The figure shows three views and two pictorial views of one solid part (mm, origin at its lowest corner). Answer the questions. Coordinates: 2 decimals unless noted, no trailing zeros. Loops run counter-clockwise (first coordinate to the right, second up) from the corner with the lowest first, then second, coordinate; pieces in that order, holes last. Notation, with made-up numbers: (46, 76) - (56, 76) arc R16 cw to (56, 81) - close; hole circle Ø8 at (0, 71.25). An arc over 180 degrees is marked (long way). Return JSON: item names as keys, results as strings. Group by question number.
1. This flat-tipped pin is pushed along its axis until it touches: P1, Ø4, axis at x = 40, y = 50, coming from the -Z side. Where does it stop, or does it pass through?
2. Section A-A (y = 5.3) is taken. Write down the section's boundary in (x, z), and give its area (3 significant figures).
3. Section B-B (x = 22.25) is taken. Write down the section's boundary in (y, z).
4. Find the intervals of material crossed by line 1 along Y through (x, z) = (22.25, 19.5); line 2 along X through (y, z) = (52.7, 18.75); line 3 along Y through (x, z) = (23, 15.5), in increasing order.
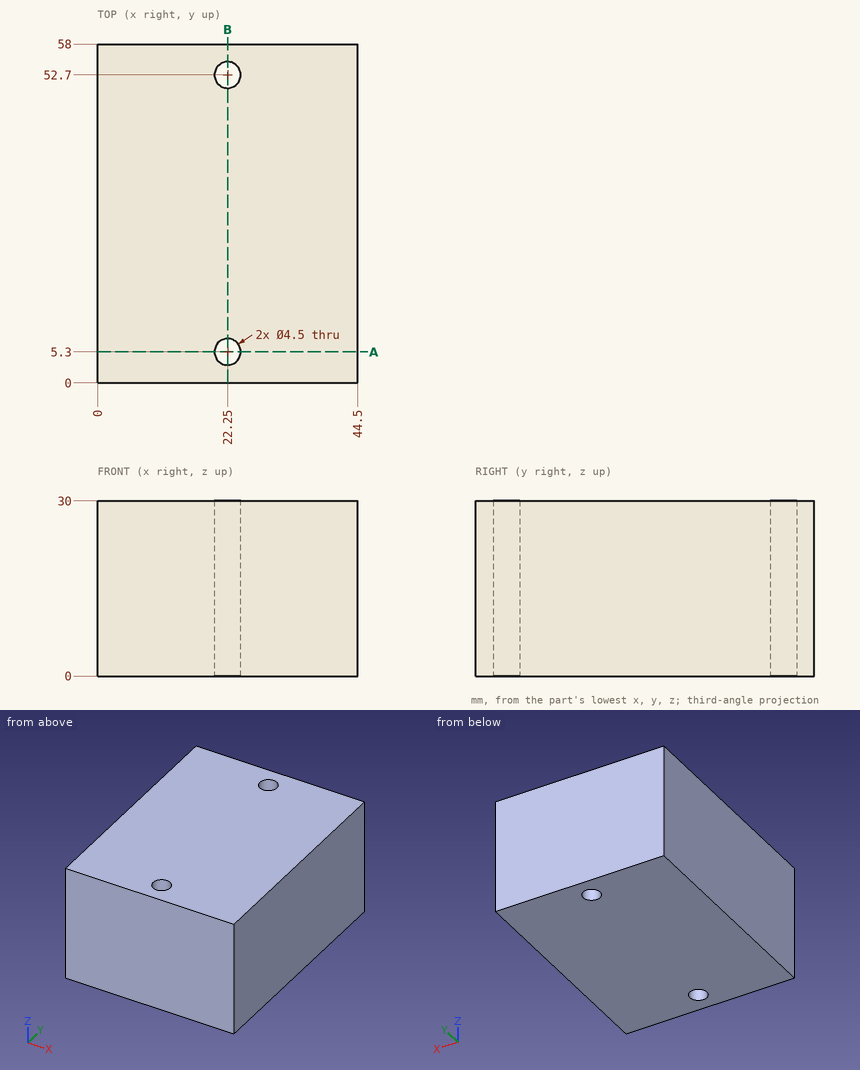
The answers:
{
 "1": {"P1": "stops at z = 0"},
 "2": {"outline": "(0, 0) - (20, 0) - (20, 30) - (0, 30) - close; (24.5, 0) - (44.5, 0) - (44.5, 30) - (24.5, 30) - close", "area": "1,200 mm2"},
 "3": {"outline": "(0, 0) - (3.05, 0) - (3.05, 30) - (0, 30) - close; (7.55, 0) - (50.45, 0) - (50.45, 30) - (7.55, 30) - close; (54.95, 0) - (58, 0) - (58, 30) - (54.95, 30) - close"},
 "4": {"line 1": "y = 0 to 3.05, 7.55 to 50.45, 54.95 to 58", "line 2": "x = 0 to 20, 24.5 to 44.5", "line 3": "y = 0 to 3.18, 7.42 to 50.58, 54.82 to 58"}
}
